Input: dimensioned drawing with shaded views. Units: mm. Origin: part minimum x, y, z. Round coordinates to 2 decimals unless told otherwise and drop trailing zeros. Loops run counter-clockwise (first coordinate to the right, second up) from the corner with the lowest first, then second, coordinate; pieces in that order, holes last. Notation, with made-up numbers: (-37.75, 48) - (21.25, 48) arc R16 cw to (21.25, 73) - close; hole circle Ø6 at (0.5, 66). An arc over 180 degrees is marked (long way). One line per question, with ' | ' between items. Start each with the question number.
Item 1: Draft query along X for the marked faces 1, 2 and 3. Return one class per face: pulls with the +X half, pulls with the -X half, needs draft (parallel to the pull), parting line crosses it, or undercut.
Item 2: Section A-A, the plane y = 46. Return loops of the section in (x, z), plus the area to 3 significant figures.
Item 3: Section B-B, the plane z = 1.85. Return loops of the section in (x, y), plus the area to 3 significant figures.
Item 4: Material intervals for line 1 along Y through (x, z) = (15, 4.05); line 2 along Y through (x, z) = (12, 2.6); line 3 along X through (y, z) = (39, 2.15), sorted ascending.
Item 5: Section C-C, the plane x = 9. Return loops of the section in (y, z), plus the area to 3 significant figures.
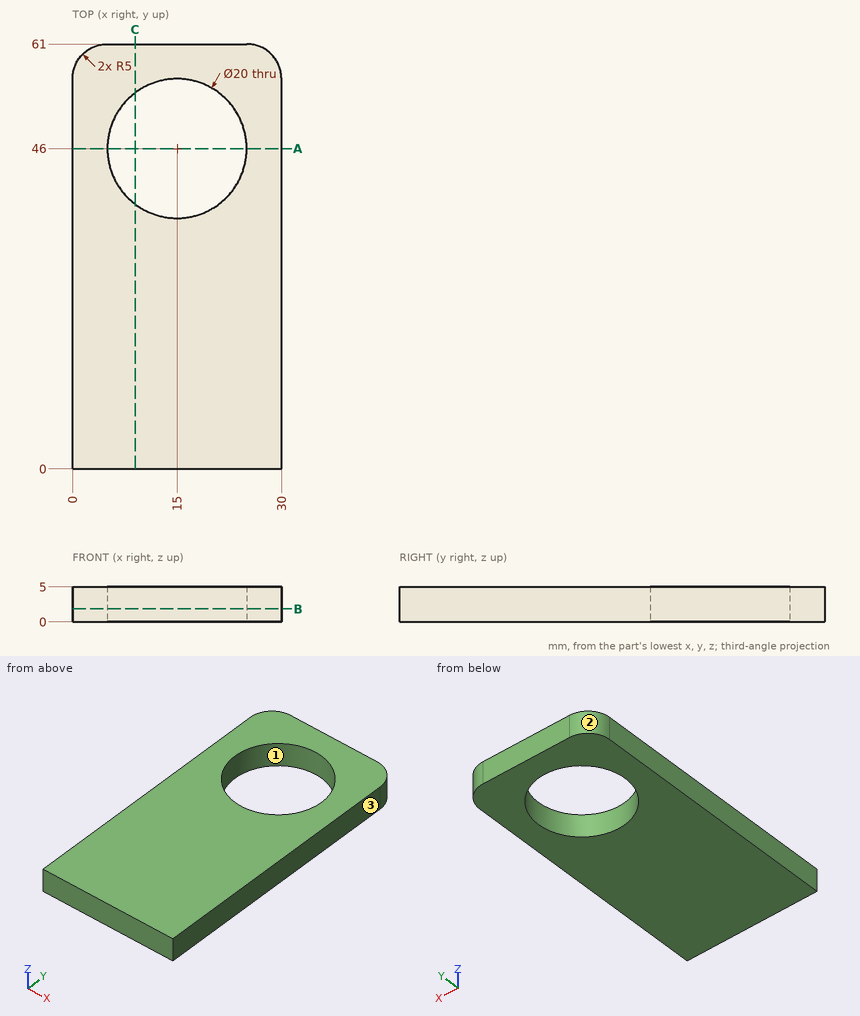
Return value:
1) face 1: undercut | face 2: pulls with the -X half | face 3: pulls with the +X half
2) outline: (0, 0) - (5, 0) - (5, 5) - (0, 5) - close; (25, 0) - (30, 0) - (30, 5) - (25, 5) - close | area: 50.0 mm2
3) outline: (0, 0) - (30, 0) - (30, 56) arc R5 ccw to (25, 61) - (5, 61) arc R5 ccw to (0, 56) - close; hole circle Ø20 at (15, 46) | area: 1,510 mm2
4) line 1: 0 to 36, 56 to 61 | line 2: 0 to 36.46, 55.54 to 61 | line 3: 0 to 7.86, 22.14 to 30
5) outline: (0, 0) - (38, 0) - (38, 5) - (0, 5) - close; (54, 0) - (61, 0) - (61, 5) - (54, 5) - close | area: 225 mm2
